```python
from build123d import *

# Parameters (mm, degrees)
SKETCH1_W           = 92.5
SKETCH1_H           = 10
SKETCH2_R           = 87.5
BOSS_EXTRUDE1_DEPTH = 100
CUT_EXTRUDE1_START  = -12
CUT_EXTRUDE1_DEPTH  = 12
CUT_EXTRUDE2_START  = -12
CUT_EXTRUDE2_DEPTH  = 12
CUT_EXTRUDE3_START  = -12
CUT_EXTRUDE3_DEPTH  = 12
CUT_EXTRUDE4_START  = -12
CUT_EXTRUDE4_DEPTH  = 12
HOLE1_D             = 135


with BuildPart() as part:
    # Sketch1 → Revolve1 (revolve)
    with BuildSketch(Plane(origin=(0, 234.743963655, 0), x_dir=(1, 0, 0), z_dir=(0, 1, 0))):
        with Locations((567.480642584, 1252.692981355)):
            Rectangle(SKETCH1_W, SKETCH1_H)
    revolve(axis=Axis((521.230642584, 234.743963655, -1257.692981355), (0, 0, 1)))

    # Sketch2 → Boss-Extrude1 (add)
    with BuildSketch(Plane(origin=(0, 0, -1257.692981355), x_dir=(-1, 0, 0), z_dir=(0, 0, -1))):
        with Locations((-521.230642584, 234.743963655)):
            Circle(SKETCH2_R)
    extrude(amount=BOSS_EXTRUDE1_DEPTH)

    # Sketch3 → Cut-Extrude1 (cut)
    with BuildSketch(Plane(origin=(0, 0, -1357.692981355), x_dir=(-1, 0, 0), z_dir=(0, 0, -1)).offset(CUT_EXTRUDE1_START)):
        with BuildLine():
            ThreePointArc((-433.971284296, 241.228899354), (-436.730642584, 234.743963655), (-433.971284296, 228.259027955))
            ThreePointArc((-433.971284296, 228.259027955), (-433.730642584, 234.743963655), (-433.971284296, 241.228899354))
        make_face()
    extrude(amount=CUT_EXTRUDE1_DEPTH, mode=Mode.SUBTRACT)

    # Sketch4 → Cut-Extrude2 (cut)
    with BuildSketch(Plane(origin=(0, 0, -1357.692981355), x_dir=(-1, 0, 0), z_dir=(0, 0, -1)).offset(CUT_EXTRUDE2_START)):
        with BuildLine():
            ThreePointArc((-514.745706884, 147.484605366), (-521.230642584, 150.243963655), (-527.715578284, 147.484605366))
            ThreePointArc((-527.715578284, 147.484605366), (-521.230642584, 147.243963655), (-514.745706884, 147.484605366))
        make_face()
    extrude(amount=CUT_EXTRUDE2_DEPTH, mode=Mode.SUBTRACT)

    # Sketch5 → Cut-Extrude3 (cut)
    with BuildSketch(Plane(origin=(0, 0, -1357.692981355), x_dir=(-1, 0, 0), z_dir=(0, 0, -1)).offset(CUT_EXTRUDE3_START)):
        with BuildLine():
            ThreePointArc((-527.715578284, 322.003321943), (-521.230642584, 319.243963655), (-514.745706884, 322.003321943))
            ThreePointArc((-514.745706884, 322.003321943), (-521.230642584, 322.243963655), (-527.715578284, 322.003321943))
        make_face()
    extrude(amount=CUT_EXTRUDE3_DEPTH, mode=Mode.SUBTRACT)

    # Sketch6 → Cut-Extrude4 (cut)
    with BuildSketch(Plane(origin=(0, 0, -1357.692981355), x_dir=(-1, 0, 0), z_dir=(0, 0, -1)).offset(CUT_EXTRUDE4_START)):
        with BuildLine():
            ThreePointArc((-608.490000873, 228.259027955), (-605.730642584, 234.743963654), (-608.490000873, 241.228899354))
            ThreePointArc((-608.490000873, 241.228899354), (-608.730642584, 234.743963654), (-608.490000873, 228.259027955))
        make_face()
    extrude(amount=CUT_EXTRUDE4_DEPTH, mode=Mode.SUBTRACT)

    # Hole1 (through all)
    with Locations(Plane.XY.offset(-1247.692981355)):
        with Locations((521.230642584, 234.743963655)):
            Hole(HOLE1_D / 2)


solid = part.part
```
Source: CAD feature listing. Evaluate the final solid. Frame: model axes, mm. A direction names the side the tool comes from. Coordinates: 2 decimals unless noted, no trailing zeros. Loops run counter-clockwise (first coordinate to the right, second up) from the corner with the lowest first, then second, coordinate; pieces in that order, holes last. Notation, with made-up numbers: M 40,-1.75 L 53,-1.75 A24 ccw 53,11.25 Z; hole C -13.75,-3 d1. An arc over 180 degrees is marked long. Use a Markdown table: item, result. Add a question column.
Q1. Section query D-D, the plane y = 306.5. Return loops of the section in (x, z).
Q2. First-contact query: pin 1 (3 mm diameter, centred on x = 540.5, z = -1345.5, fed in from -Y); pin 2 (0.9 mm diameter, centred on x = 519.5, y = 321, fed in from -Z); pin 3 (3 mm diameter, centred on x = 560, z = -1265, fed in from +Y). Flat tips, straight axial feed; report the tip coordinate or a pass-through.
Q3. Section query A-A, the plane y = 179.5. Return loops of the section in (x, z), and give its area (3 significant figures).
Q4. Access query for faces 1 (the cylindrical face through (605.73, 234.64, -1351.61)), 2 (the flat face through (484, 178, -1357.693)), 3 (the cylindrical face through (521.129, 150.243, -1351.609)), 4 (the flat face through (576.5, 166.7, -1257.693)). Directions: +Z, -Z, +X, -X, +Y, -Y. A direction counts if a zero-diameter tool reaches every point of the face in a straight line with its end or side. Return the directions, or none.
Q5. Section query B-B, the plane x = 518. Return loops of the section in (y, z), and give its area (3 significant figures).
Q6. Draft query along Y for faces 5 (the cylindrical face through (458.88, 208.89, -1303.46)), 6 (the cylindrical face through (436.73, 234.85, -1351.61)), 7 (the flat face through (515, 167, -1247.693)), 8 (the cylindrical face through (521.332, 319.245, -1351.609)). Return one class per face: pulls with the +Y half, pulls with the -Y half, needs draft (parallel to the pull), parting line crosses it, or undercut.
Q7. Material intervals for L1, parallel to Y at x = 538.5, z = -1289.5; L2, parallel to X at y = 271.5, z = -1257.5; L3, parallel to X at y = 174, z = -1305, sorted ascending.
Q8. Section query C-C, the plane z = -1348. Return loops of the section in (x, y).
Result:
| question | item | result |
|---|---|---|
| 1 | outline | M 462.86,-1257.69 L 471.16,-1257.69 L 471.16,-1357.69 L 571.3,-1357.69 L 571.3,-1257.69 L 579.6,-1257.69 L 579.6,-1247.69 L 462.86,-1247.69 Z |
| 2 | pin 1 | stops at y = 149.07 |
| 2 | pin 2 | stops at z = -1345.69 |
| 2 | pin 3 | stops at y = 313.91 |
| 3 | outline | M 447.04,-1257.69 L 453.38,-1257.69 L 453.38,-1357.69 L 482.44,-1357.69 L 482.44,-1247.69 L 447.04,-1247.69 Z; M 560.02,-1357.69 L 589.09,-1357.69 L 589.09,-1257.69 L 595.42,-1257.69 L 595.42,-1247.69 L 560.02,-1247.69 Z |
| 3 | area | 6,520 mm2 |
| 4 | face 1 | -Z, +X |
| 4 | face 2 | -Z, +X, -X, +Y, -Y |
| 4 | face 3 | -Z, -Y |
| 4 | face 4 | -Z |
| 5 | outline | M 142.3,-1257.69 L 147.3,-1257.69 L 147.3,-1345.69 L 149.64,-1345.69 L 149.64,-1357.69 L 167.32,-1357.69 L 167.32,-1247.69 L 142.3,-1247.69 Z; M 302.17,-1357.69 L 319.84,-1357.69 L 319.84,-1345.69 L 322.18,-1345.69 L 322.18,-1257.69 L 327.19,-1257.69 L 327.19,-1247.69 L 302.17,-1247.69 Z |
| 5 | area | 4,450 mm2 |
| 6 | face 5 | undercut |
| 6 | face 6 | undercut |
| 6 | face 7 | needs draft |
| 6 | face 8 | pulls with the +Y half |
| 7 | L1 | y = 148.97 to 169.49, 300 to 320.52 |
| 7 | L2 | x = 436.35 to 464.62, 577.85 to 606.11 |
| 7 | L3 | x = 458.25 to 491.8, 550.67 to 584.21 |
| 8 | outline | M 433.97,228.26 A87.5 ccw 514.75,147.48 A9 cw 527.72,147.48 A87.5 ccw 608.49,228.26 A9 cw 608.49,241.23 A87.5 ccw 527.72,322 A9 cw 514.75,322 A87.5 ccw 433.97,241.23 A9 cw Z; hole C 521.23,234.74 d135 |
